Part model, mm, in its own coordinate system. A direction names the side the tool comes from. Coordinates: 2 decimals unless noted, no trailing zeros. Loops run counter-clockwise (first coordinate to the right, second up) from the corner with the lowest first, then second, coordinate; pieces in that order, holes last. Notation, with made-up numbers: (81.5, 16.25) - (134.5, 16.25) arc R10 ccw to (134.5, 29.25) - close; hole circle Ø10 at (-14, 84). An arc over 180 degrees is marked (long way). Use a Markdown table: item, result. Add a question column.
1) Probe probe 1 along Y at (x, z) = (4, 3.75); probe 2 along Z at (x, y) = (5.25, 4.75); probe 3 along Z at (x, y) = (-2.75, 12.75). List the from-to ranges inside material, lowest first. Write a range as [from, to].
2) Band-saw the part on D-D (y = 2.5). Give the cut face in (x, z), plus the area to 3 significant figures.
3) Band-saw the part on B-B (x = 0). Give the cut face in (y, z).
4) Tool access for faces 1 (the face through (0, 0, 0)), 2 (the face through (-5, 5, -2)): list every direction of +Z, -Z, +X, -X, +Y, -Y with a clear straight run to the whole face (end or side of a thin tool).
5) Band-saw the part on C-C (y = 8.25). Give the cut face in (x, z).
6) Band-saw the part on A-A (z = 0). Give the cut face in (x, y).
7) Drop flat-ended pins along their axis: P1, Ø4, axis at y = 11.5, z = -5, coming from the +X side; P2, Ø4, axis at y = 10, z = 4.5, coming from the -X side; P3, Ø1, axis at x = -3.5, y = 13, coming from the +Z side; P4, Ø4, axis at x = -4.5, z = -1, coming from the -Y side. Give the stop position or say it passes through.
from build123d import *

# Parameters (mm, degrees)
CHAMFER1_SIZE = 0.5


with BuildPart() as part:
    # Sketch1 → Revolve1 (revolve)
    with BuildSketch(Plane(origin=(0, 0, 0), x_dir=(0, 0, -1), z_dir=(1, 0, 0))):
        Polygon((0, 15), (5, 15), (5, 5), (7.5, 5), (7.5, 0), (0, 0), align=None)
    revolve(axis=Axis((0, 0, 0), (0, 1, 0)))

    # Chamfer1
    chamfer1_edges = [part.edges().sort_by_distance(p)[0] for p in [
        (0, 0, 7.5),
        (0, 5, 7.5),
        (0, 15, 5),
    ]]
    chamfer(chamfer1_edges, length=CHAMFER1_SIZE)


solid = part.part
Answer block:
| question | item | result |
|---|---|---|
| 1 | probe 1 | [0, 5] |
| 1 | probe 2 | [-5, 5] |
| 1 | probe 3 | [-4.18, 4.18] |
| 2 | outline | circle Ø15 at (0, 0) |
| 2 | area | 177 mm2 |
| 3 | outline | (0, -7) - (0.5, -7.5) - (4.5, -7.5) - (5, -7) - (5, -5) - (14.5, -5) - (15, -4.5) - (15, 4.5) - (14.5, 5) - (5, 5) - (5, 7) - (4.5, 7.5) - (0.5, 7.5) - (0, 7) - close |
| 4 | face 1 | +Z, -Z, +X, -X, -Y |
| 4 | face 2 | +Y |
| 5 | outline | circle Ø10 at (0, 0) |
| 6 | outline | (-7.5, 0.5) - (-7, 0) - (7, 0) - (7.5, 0.5) - (7.5, 4.5) - (7, 5) - (5, 5) - (5, 14.5) - (4.5, 15) - (-4.5, 15) - (-5, 14.5) - (-5, 5) - (-7, 5) - (-7.5, 4.5) - close |
| 7 | P1 | x = 4 |
| 7 | P2 | x = -4.33 |
| 7 | P3 | z = 4 |
| 7 | P4 | y = 0 |
